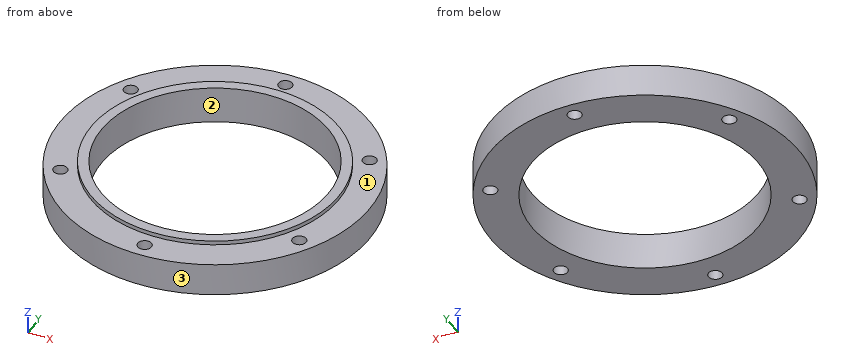
from build123d import *

# Parameters (mm, degrees)
SKETCH1_R           = 75
SKETCH1_R_2         = 55
SKETCH1_R_3         = 3.325
BOSS_EXTRUDE1_DEPTH = 16
SKETCH2_R           = 60
SKETCH2_R_2         = 55
BOSS_EXTRUDE2_DEPTH = 2


with BuildPart() as part:
    # Sketch1 → Boss-Extrude1 (new body)
    with BuildSketch(Plane.XY):
        Circle(SKETCH1_R)
        Circle(SKETCH1_R_2, mode=Mode.SUBTRACT)
        with Locations((0, 67.5)):
            Circle(SKETCH1_R_3, mode=Mode.SUBTRACT)
        with Locations((58.456714755, 33.75)):
            Circle(SKETCH1_R_3, mode=Mode.SUBTRACT)
        with Locations((58.456714755, -33.75)):
            Circle(SKETCH1_R_3, mode=Mode.SUBTRACT)
        with Locations((0, -67.5)):
            Circle(SKETCH1_R_3, mode=Mode.SUBTRACT)
        with Locations((-58.456714755, -33.75)):
            Circle(SKETCH1_R_3, mode=Mode.SUBTRACT)
        with Locations((-58.456714755, 33.75)):
            Circle(SKETCH1_R_3, mode=Mode.SUBTRACT)
    extrude(amount=BOSS_EXTRUDE1_DEPTH)

    # Sketch2 → Boss-Extrude2 (add)
    with BuildSketch(Plane.XY.offset(16)):
        Circle(SKETCH2_R)
        Circle(SKETCH2_R_2, mode=Mode.SUBTRACT)
    extrude(amount=BOSS_EXTRUDE2_DEPTH)


solid = part.part
Can you work these out from the model? Positions are in its coordinate system, mm. Face numbers are marked on the shaded views. Coordinates: 2 decimals unless noted, no trailing zeros. Write each loop counter-clockwise with the first axis right and the second up, starting at its lowest first coordinate (ties: lowest second). Pieces come first, ordered by that corner, then holes.
Q1. If we mould it in two halves opening along X, with no side actions, what happens to the marked faces 1, 2 and 3? For each: +X half, -X half, draft (parallel to the pull), parting line (faces both ways), or undercut.
Results found:
face 1: draft
face 2: undercut
face 3: parting line
Q2. Imagine slicing it at C-C, the plane z = 3.25. List the corners of the cut face in (x, y) for me (3 decimals).
Results found:
outline: circle Ø150 at (0, 0); hole circle Ø6.65 at (-58.457, -33.75); hole circle Ø6.65 at (-58.457, 33.75); hole circle Ø110 at (0, 0); hole circle Ø6.65 at (0, -67.5); hole circle Ø6.65 at (0, 67.5); hole circle Ø6.65 at (58.457, -33.75); hole circle Ø6.65 at (58.457, 33.75)
Q3. Imagine slicing it at D-D, the plane x = 48. List the corners of the cut face in (y, z) for me.
Results found:
outline: (-57.63, 0) - (-26.85, 0) - (-26.85, 18) - (-36, 18) - (-36, 16) - (-57.63, 16) - close; (26.85, 0) - (57.63, 0) - (57.63, 16) - (36, 16) - (36, 18) - (26.85, 18) - close
Q4. For P1, Ø3, axis at y = 32.5, z = 14, coming from the +X side; P2, Ø4, axis at y = -59, z = 13, coming from the -X side; P3, Ø1.5, axis at x = -42.5, z = 7.5, coming from the -Y side; P4, Ø10.5, axis at x = -58.46, y = -33.75, coming from the -Z side, each with a flat end and sliding along its axis, tell me the tip position at first contact or that it passes through.
Results found:
P1: stops at x = 68.29
P2: stops at x = -48.74
P3: stops at y = -62.31
P4: stops at z = 0
Q5. Imagine slicing it at B-B, the plane y = 51. List the corners of the cut face in (x, z) for me, plus the area to 3 significant figures.
Results found:
outline: (-54.99, 0) - (-20.59, 0) - (-20.59, 18) - (-31.61, 18) - (-31.61, 16) - (-54.99, 16) - close; (20.59, 0) - (54.99, 0) - (54.99, 16) - (31.61, 16) - (31.61, 18) - (20.59, 18) - close
area: 1,140 mm2
Q6. Please list where these lines run through material, in increasing order: L1, parallel to Y at x = 0, z = 11.25 (3 decimals); L2, parallel to Y at x = -59, z = 9.5; L3, parallel to Z at x = -43.5, y = 44.5.
Results found:
L1: y = -75 to -70.825, -64.175 to -55, 55 to 64.175, 70.825 to 75
L2: y = -46.3 to -37.03, -30.47 to 30.47, 37.03 to 46.3
L3: z = 0 to 16
Q7. Imagine slicing it at A-A, the plane x = 0. List the corners of the cut face in (y, z) for me (3 decimals), plus the area to 3 significant figures.
Results found:
outline: (-75, 0) - (-70.825, 0) - (-70.825, 16) - (-75, 16) - close; (-64.175, 0) - (-55, 0) - (-55, 18) - (-60, 18) - (-60, 16) - (-64.175, 16) - close; (55, 0) - (64.175, 0) - (64.175, 16) - (60, 16) - (60, 18) - (55, 18) - close; (70.825, 0) - (75, 0) - (75, 16) - (70.825, 16) - close
area: 447 mm2
